Build history of the part. All positions in model axes, mm. A direction names the side the tool comes from. Round coordinates to 2 decimals unless told otherwise and drop trailing zeros. Write each loop counter-clockwise with the first axis right and the second up, starting at its lowest first coordinate (ties: lowest second). Pieces come first, ordered by that corner, then holes. Notation, with made-up numbers: (32.5, 41.5) - (66.5, 41.5) arc R36 cw to (66.5, 78.5) - close; hole circle Ø11 at (69.5, -23). An arc over 180 degrees is marked (long way). Answer as a JSON object with one key per item and string values. Group by question number.
Item 1: Slice it at B-B, the plane z = 5.7. List the corners of the cut face in (x, y) (3 decimals), then the cut area to 3 significant figures.
Item 2: Which spindle directions (+Z, -Z, +X, -X, +Y, -Y) get a long thin tool onto all of the face, cutting with end or side? Do faces 5 (the flat face through (0, 5, 0)), 6 (the cylindrical face through (-3.33, 2.26, 2.96)), 7 (the cylindrical face through (-8.76, 2.26, 2.97)), 8 (the cylindrical face through (8.76, 6.98, 7.97)). Say none if no direction does.
Item 3: Flat gauge pins, fed straight in: pin 1 (3 mm diameter, centred on x = 6.075, z = 0.2, fed in from -Y); pin 2 (3 mm diameter, centred on x = 4.5, z = 5.5, fed in from -Y); pin 3 (1.4 mm diameter, centred on x = 1, y = 2.5, fed in from +Z); pin 4 (1 mm diameter, centred on y = 3, z = 3, fed in from +X). Where does each tip first touch, or does it go through?
Item 4: Slice it at A-A, the plane y = 6.95. List the corners of the cut face in (x, z) (3 decimals), then the cut area to 3 significant figures.
Item 5: Slice it at C-C, the plane x = 5.25. List the corners of the cut face in (y, z) (3 decimals).
Item 6: Two-plate mould, pull along X, no slides. Class faces 1 (the flat face through (-3.1, 6, 3)), 2 (the flat face through (6, 2, 3.2)), 3 (the cylindrical face through (3.33, 6.98, 7.96)), 4 (the cylindrical face through (8.77, 2.26, 2.96)): +X half, -X half, draft (parallel to the pull), parting line (faces both ways), or undercut.
Item 7: Probe line 1 (X direction, y = 2, z = 1.5); line 2 (Y direction, x = 7.1, z = 5.7) (3 decimals); line 3 (X direction, y = 5.5, z = 0.75). List the from-to ranges inside material, lowest first. Write a range as from..to.
Item 8: Slice it at D-D, the plane y = 4. List the corners of the cut face in (x, z) (3 decimals), then the cut area to 3 significant figures.
from build123d import *

# Parameters (mm, degrees)
EXTRUDE_1_DEPTH     = 4.45
EXTRUDE_2_DEPTH     = 5
HOLE_WIZARD_M3_1_D  = 2.5
SKETCH_5_R          = 1.525
CUT_EXTRUDE_1_DEPTH = 22.921279616
FILLET_R0_8_1_R     = 0.8


with BuildPart() as part:
    # 草图1 → 凸台-拉伸1 (new body)
    with BuildSketch(Plane(origin=(0, 0, 0), x_dir=(1, 0, 0), z_dir=(0, 1, 0))):
        Polygon((-9, 2.8), (9, 2.8), (9, -3.2), (3.1, -3.2), (3.1, 0), (-3.1, 0), (-3.1, -3.2), (-9, -3.2), align=None)
    extrude(amount=EXTRUDE_1_DEPTH)

    # 草图2 → 凸台-拉伸2 (add)
    with BuildSketch(Plane(origin=(0, 4.45, 0), x_dir=(1, 0, 0), z_dir=(0, 1, 0))):
        Polygon((-3.1, -8.2), (-3.1, 0), (3.1, 0), (3.1, -8.2), (9, -8.2), (9, 2.8), (-9, 2.8), (-9, -8.2), align=None)
    extrude(amount=EXTRUDE_2_DEPTH)

    # M3 螺纹孔1 (through all)
    with Locations(Plane.XZ):
        with Locations((-6.075, 0.2), (6.075, 0.2)):
            Hole(HOLE_WIZARD_M3_1_D / 2)

    # 草图5 → 切除-拉伸1 (cut, through all)
    with BuildSketch(Plane.ZY.offset(9)):
        with Locations((5.7, 6.95)):
            Circle(SKETCH_5_R)
    extrude(amount=-CUT_EXTRUDE_1_DEPTH, mode=Mode.SUBTRACT)

    # R0.8 圆角1
    fillet_r0_8_1_edges = [part.edges().sort_by_distance(p)[0] for p in [
        (-9, 4.725, -2.8),
        (9, 4.725, -2.8),
        (9, 2.225, 3.2),
        (3.1, 2.225, 3.2),
        (3.1, 4.725, 0),
        (-3.1, 4.725, 0),
        (-3.1, 2.225, 3.2),
        (-9, 2.225, 3.2),
        (-9, 6.95, 8.2),
        (-3.1, 6.95, 8.2),
        (3.1, 6.95, 8.2),
        (9, 6.95, 8.2),
    ]]
    fillet(fillet_r0_8_1_edges, radius=FILLET_R0_8_1_R)


solid = part.part
Geometry says:
{
 "1": {"outline": "(-9, 4.45) - (-3.1, 4.45) - (-3.1, 5.425) - (-9, 5.425) - close; (-9, 8.475) - (-3.1, 8.475) - (-3.1, 9.45) - (-9, 9.45) - close; (3.1, 4.45) - (9, 4.45) - (9, 5.425) - (3.1, 5.425) - close; (3.1, 8.475) - (9, 8.475) - (9, 9.45) - (3.1, 9.45) - close", "area": "23.0 mm^2"},
 "2": {"face 5": "+Z, +Y, -Y", "face 6": "+Z, -Y", "face 7": "+Z, -X, -Y", "face 8": "+Z, +X, +Y, -Y"},
 "3": {"pin 1": "stops at y = 0", "pin 2": "stops at y = 4.45", "pin 3": "stops at z = 0", "pin 4": "stops at x = 8.99"},
 "4": {"outline": "(-9, -2) arc R0.8 ccw to (-8.2, -2.8) - (8.2, -2.8) arc R0.8 ccw to (9, -2) - (9, 4.175) - (3.1, 4.175) - (3.1, 0.8) arc R0.8 cw to (2.3, 0) - (-2.3, 0) arc R0.8 cw to (-3.1, 0.8) - (-3.1, 4.175) - (-9, 4.175) - close; (-9, 7.225) - (-3.1, 7.225) - (-3.1, 7.4) arc R0.8 ccw to (-3.9, 8.2) - (-8.2, 8.2) arc R0.8 ccw to (-9, 7.4) - close; (3.1, 7.225) - (9, 7.225) - (9, 7.4) arc R0.8 ccw to (8.2, 8.2) - (3.9, 8.2) arc R0.8 ccw to (3.1, 7.4) - close; hole circle Ø2.5 at (-6.075, 0.2); hole circle Ø2.5 at (6.075, 0.2)", "area": "101 mm^2"},
 "5": {"outline": "(0, -2.8) - (9.45, -2.8) - (9.45, -0.739) - (0, -0.739) - close; (0, 1.139) - (9.45, 1.139) - (9.45, 8.2) - (4.45, 8.2) - (4.45, 3.2) - (0, 3.2) - close; hole circle Ø3.05 at (6.95, 5.7)"},
 "6": {"face 1": "undercut", "face 2": "draft", "face 3": "undercut", "face 4": "+X half"},
 "7": {"line 1": "x = -9..-3.1, 3.1..9", "line 2": "y = 4.45..5.425, 8.475..9.45", "line 3": "x = -9..-7.2, -4.95..-3.1, 3.1..4.95, 7.2..9"},
 "8": {"outline": "(-9, -2) arc R0.8 ccw to (-8.2, -2.8) - (8.2, -2.8) arc R0.8 ccw to (9, -2) - (9, 2.4) arc R0.8 ccw to (8.2, 3.2) - (3.9, 3.2) arc R0.8 ccw to (3.1, 2.4) - (3.1, 0.8) arc R0.8 cw to (2.3, 0) - (-2.3, 0) arc R0.8 cw to (-3.1, 0.8) - (-3.1, 2.4) arc R0.8 ccw to (-3.9, 3.2) - (-8.2, 3.2) arc R0.8 ccw to (-9, 2.4) - close; hole circle Ø2.5 at (-6.075, 0.2); hole circle Ø2.5 at (6.075, 0.2)", "area": "77.8 mm^2"}
}
